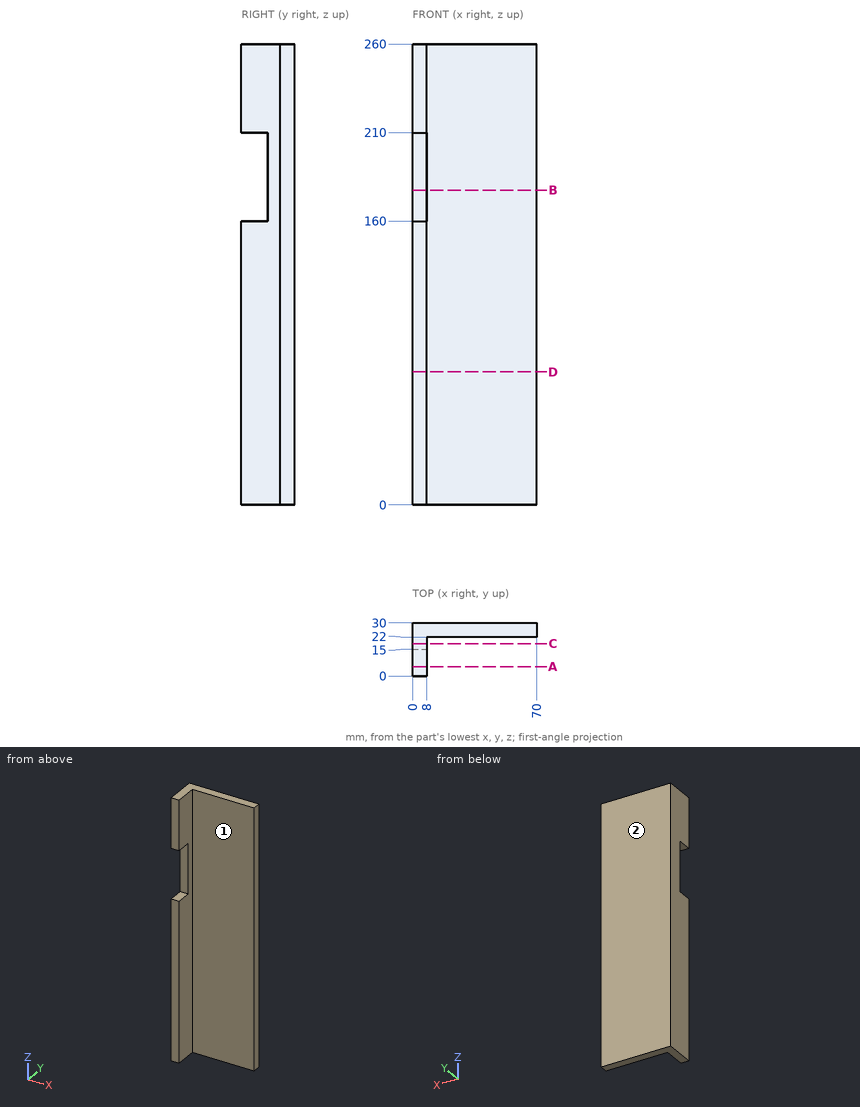
Design review of the part shown in the three views and the two pictorial views. Dimensions are in mm from the part's minimum x, y and z. A direction names the side the tool comes from. Give positions to 0.01 mm unless a question says otherwise; leave off trailing zeros. Loops run counter-clockwise (first coordinate to the right, second up) from the corner with the lowest first, then second, coordinate; pieces in that order, holes last. Notation, with made-up numbers: (78.25, 65) -> (87.25, 65) arc R24 cw to (87.25, 101) -> close; hole circle Ø5 at (26, 46). An arc over 180 degrees is marked (long way). Write each question's results on one line, items separated by ' | '.
1) For line 1 along Z through (x, y) = (3, 4); line 2 along X through (y, z) = (3, 101); line 3 along Y through (x, z) = (28, 130), list the stretches that pass through material, from the lowest coordinate up. Write a range as from..to.
Conclusion:
line 1: z = 0..160, 210..260 | line 2: x = 0..8 | line 3: y = 22..30
2) Take a section at B-B, the plane z = 177.5. Give the boundary of the cut face in (x, y), plus the area to 3 significant figures.
Conclusion:
outline: (0, 15) -> (8, 15) -> (8, 22) -> (70, 22) -> (70, 30) -> (0, 30) -> close | area: 616 mm^2
3) Insertion check: pin 1 Ø6.5 at (x, z) = (5, 186.5) entering from -Y; pin 2 Ø1.5 at (x, z) = (48.5, 208) entering from -Y; pin 3 Ø5 at (y, z) = (17, 129.5) entering from +X. Each pin has a flat end and moves straight along its axis. Give the tip position at first contact, or say it passes through.
Conclusion:
pin 1: stops at y = 15 | pin 2: stops at y = 22 | pin 3: stops at x = 8
4) Take a section at C-C, the plane y = 18.25. Give the boundary of the cut face in (x, z).
Conclusion:
outline: (0, 0) -> (8, 0) -> (8, 260) -> (0, 260) -> close
5) Tool access review of the marked faces 1 and 2: name each direction out of +Z, -Z, +X, -X, +Y, -Y from which nothing blocks a thin tool from reaching the whole face with its end or side.
Conclusion:
face 1: +Z, -Z, +X, -Y | face 2: +Z, -Z, +X, -X, +Y
6) Take a section at A-A, the plane y = 5.25. Give the boundary of the cut face in (x, z).
Conclusion:
outline: (0, 0) -> (8, 0) -> (8, 160) -> (0, 160) -> close; (0, 210) -> (8, 210) -> (8, 260) -> (0, 260) -> close
7) Take a section at D-D, the plane z = 75. Give the boundary of the cut face in (x, y).
Conclusion:
outline: (0, 0) -> (8, 0) -> (8, 22) -> (70, 22) -> (70, 30) -> (0, 30) -> close
